Can you work these out from the drawing? Everything is in mm from the part's minimum corner. A direction names the side the tool comes from. Coordinates: 2 decimals unless noted, no trailing zeros. Loops run counter-clockwise (first coordinate to the right, second up) from the corner with the lowest first, then second, coordinate; pieces in that order, holes last.
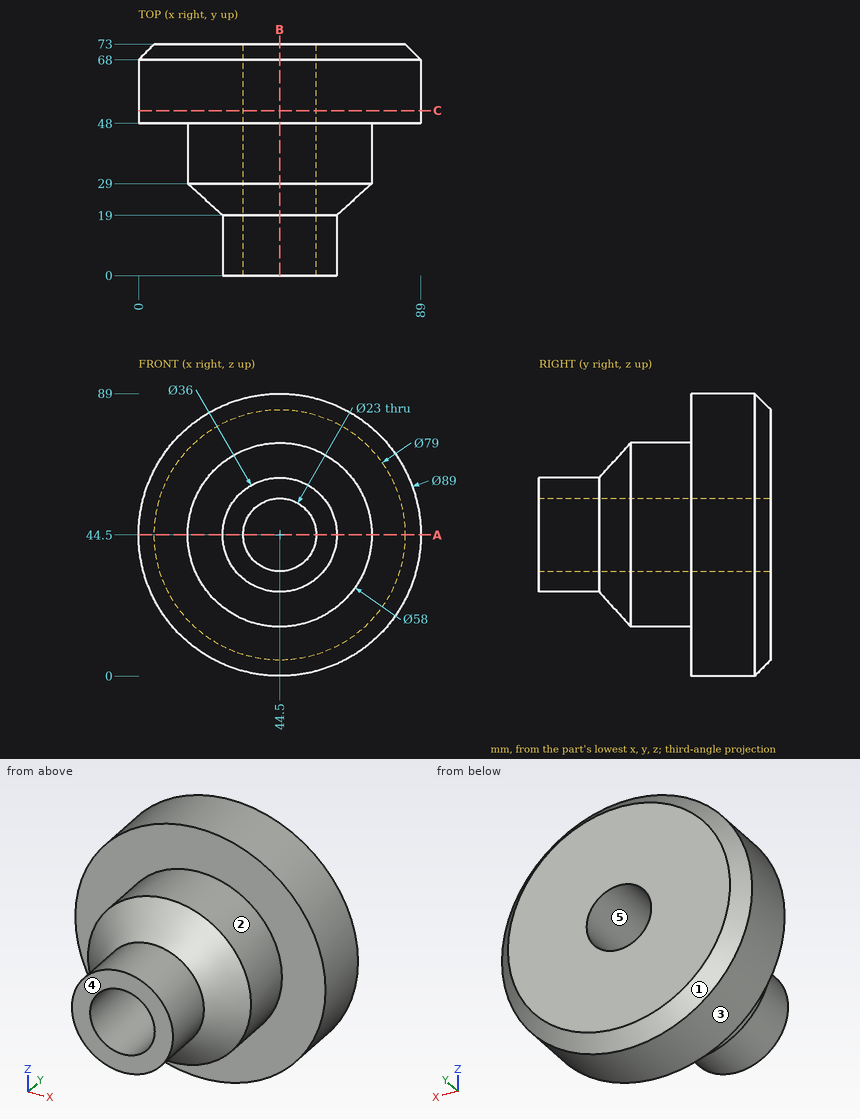
Item 1: I'm going to push flat-ended pins straight in: P1, Ø10, axis at y = 58.5, z = 74.5, coming from the -X side; P2, Ø8, axis at x = 18.5, z = 38, coming from the -Y side; P3, Ø1.5, axis at y = 33.5, z = 61, coming from the -X side. Where does each tip first touch, or does it pass through?
Results are:
P1: stops at x = 7.69
P2: stops at y = 23.36
P3: stops at x = 20.15
Item 2: Suppose I cut it at A-A, the plane z = 44.5. Please give me the cut outline in (x, y), plus the area to 3 significant figures.
Results are:
outline: (0, 48) - (15.5, 48) - (15.5, 29) - (26.5, 19) - (26.5, 0) - (33, 0) - (33, 73) - (5, 73) - (0, 68) - close; (56, 0) - (62.5, 0) - (62.5, 19) - (73.5, 29) - (73.5, 48) - (89, 48) - (89, 68) - (84, 73) - (56, 73) - close
area: 2,780 mm2
Item 3: Suppose I cut it at C-C, the plane y = 52. Please give me the cut outline in (x, z), plus the area to 3 significant figures.
Results are:
outline: circle Ø89 at (44.5, 44.5); hole circle Ø23 at (44.5, 44.5)
area: 5,810 mm2
Item 4: I need wall thicknesses on line 1 along X through (y, z) = (49.5, 44.5); line 2 along X through (y, z) = (30, 44). Which ranges of each line are inside material? Lowest first, please.
Results are:
line 1: x = 0 to 33, 56 to 89
line 2: x = 15.5 to 33.01, 55.99 to 73.5
Item 5: On a 3-axis mill with a long thin cutter (end or side, diameter ignored), from which of +Z, -Z, +X, -X, +Y, -Y can I reach the whole of each face in a straight line? I mean the marked faces 1 and 2. Say none if no direction works.
Results are:
face 1: +Y
face 2: -Y
Item 6: We'd pull the mould along X, two halves only. Please class the marked faces 3, 4 and 5: +X half, -X half, draft (parallel to the pull), parting line (faces both ways), or undercut.
Results are:
face 3: parting line
face 4: draft
face 5: undercut
Item 7: Suppose I cut it at B-B, the plane x = 44.5. Please give me the cut outline in (y, z), plus the area to 3 significant figures.
Results are:
outline: (0, 26.5) - (19, 26.5) - (29, 15.5) - (48, 15.5) - (48, 0) - (68, 0) - (73, 5) - (73, 33) - (0, 33) - close; (0, 56) - (73, 56) - (73, 84) - (68, 89) - (48, 89) - (48, 73.5) - (29, 73.5) - (19, 62.5) - (0, 62.5) - close
area: 2,780 mm2
